from build123d import *

# Parameters (mm, degrees)
YOKE_BODY_DEPTH           = 23
TOP_BLOCK_DEPTH           = 10
TOP_BORE_SKETCH_R         = 8
TOP_BORE_16_DEPTH         = 130.533779378
TOP_COLLAR_SKETCH_R       = 18
TOP_COLLAR_36_DEPTH       = 5
COLLAR_BORE_20_REACH      = 122.147
COLLAR_BORE_SKETCH_R      = 10
SIDE_PIVOT_BOSS_SKETCH_R  = 13
SIDE_PIVOT_BOSS_26_DEPTH  = 19
SIDE_PIVOT_BORE_SKETCH_R  = 6
SIDE_PIVOT_BORE_12_DEPTH  = 130.206230518
SUPPORT_RIB_REACH         = 108.584
SUPPORT_RIB_SKETCH_WALL_W = 247.172853136
SUPPORT_RIB_SKETCH_WALL_H = 10


with BuildPart() as part:
    # Yoke Profile Sketch → Yoke Body (new, symmetric)
    with BuildSketch(Plane.XY):
        with BuildLine():
            Line((19, 10), (-19, 10))
            ThreePointArc((-19, 10), (-21.828427125, 8.828427125), (-23, 6))
            Line((-23, 6), (-23, -21.741149913))
            ThreePointArc((-23, -21.741149913), (-23.246067912, -23.290385113), (-23.960051881, -24.687133484))
            Line((-23.960051881, -24.687133484), (-41.539948119, -48.795166343))
            ThreePointArc((-41.539948119, -48.795166343), (-42.253932088, -50.191914714), (-42.5, -51.741149913))
            Line((-42.5, -51.741149913), (-42.5, -71.741149913))
            Line((-42.5, -71.741149913), (-32.5, -71.741149913))
            Line((-32.5, -71.741149913), (-32.5, -55))
            ThreePointArc((-32.5, -55), (-32.253932088, -53.4507648), (-31.539948119, -52.054016429))
            Line((-31.539948119, -52.054016429), (-15.880155644, -30.579100626))
            ThreePointArc((-15.880155644, -30.579100626), (-13.738203736, -26.388855512), (-13, -21.741149913))
            Line((-13, -21.741149913), (-13, 0))
            Line((-13, 0), (13, 0))
            Line((13, 0), (13, -21.741149913))
            ThreePointArc((13, -21.741149913), (13.738203736, -26.388855512), (15.880155644, -30.579100626))
            Line((15.880155644, -30.579100626), (31.539948119, -52.054016429))
            ThreePointArc((31.539948119, -52.054016429), (32.253932088, -53.4507648), (32.5, -55))
            Line((32.5, -55), (32.5, -71.741149913))
            Line((32.5, -71.741149913), (42.5, -71.741149913))
            Line((42.5, -71.741149913), (42.5, -55))
            ThreePointArc((42.5, -55), (41.761796264, -50.352294401), (39.619844356, -46.162049287))
            Line((39.619844356, -46.162049287), (23.960051881, -24.687133484))
            ThreePointArc((23.960051881, -24.687133484), (23.246067912, -23.290385113), (23, -21.741149913))
            Line((23, -21.741149913), (23, 6))
            ThreePointArc((23, 6), (21.828427125, 8.828427125), (19, 10))
        make_face()
    extrude(amount=YOKE_BODY_DEPTH, both=True)

    # Top Block Sketch → Top Block (add)
    with BuildSketch(Plane(origin=(42.5, 0, 0), x_dir=(0, 0, -1), z_dir=(1, 0, 0))):
        with BuildLine():
            Line((-3, -95), (3, -95))
            ThreePointArc((3, -95), (17.142135624, -89.142135624), (23, -75))
            Line((23, -75), (23, -71.741149913))
            Line((23, -71.741149913), (-23, -71.741149913))
            Line((-23, -71.741149913), (-23, -75))
            ThreePointArc((-23, -75), (-17.142135624, -89.142135624), (-3, -95))
        make_face()
    top_block = extrude(amount=-TOP_BLOCK_DEPTH)

    # Top Block Mirror: Top Block across plane
    add(top_block.mirror(Plane(origin=(0, 0, 0), x_dir=(0, 0, 1), z_dir=(1, 0, 0))))

    # Top Bore Sketch → Top Bore Ø16 (cut, through all)
    with BuildSketch(Plane(origin=(42.5, 0, 0), x_dir=(0, 0, -1), z_dir=(1, 0, 0))):
        with Locations(Location((0, -75, 0), (0, 0, 90))):
            Circle(TOP_BORE_SKETCH_R)
    extrude(amount=-TOP_BORE_16_DEPTH, mode=Mode.SUBTRACT)

    # Top Collar Sketch → Top Collar Ø36 (add)
    with BuildSketch(Plane(origin=(0, 10, 0), x_dir=(1, 0, 0), z_dir=(0, 1, 0))):
        with Locations(Location((0, 0, 0), (0, 0, 90))):
            Circle(TOP_COLLAR_SKETCH_R)
    extrude(amount=TOP_COLLAR_36_DEPTH)

    # Collar Bore Sketch → Collar Bore Ø20 (cut, up to next)
    with BuildSketch(Plane(origin=(0, 15, 0), x_dir=(1, 0, 0), z_dir=(0, 1, 0)), mode=Mode.PRIVATE) as collar_bore_20_sk1:
        with Locations(Location((0, 0, 0), (0, 0, 270))):
            Circle(COLLAR_BORE_SKETCH_R)
    collar_bore_20_tool1 = extrude(collar_bore_20_sk1.sketch, amount=-COLLAR_BORE_20_REACH, mode=Mode.PRIVATE) & part.part
    add(collar_bore_20_tool1.solids().sort_by_distance((0, 15, 0))[0], mode=Mode.SUBTRACT)

    # Side Pivot Boss Sketch → Side Pivot Boss Ø26 (add)
    with BuildSketch(Plane(origin=(23, 0, 0), x_dir=(0, 0, -1), z_dir=(1, 0, 0))):
        with Locations(Location((0, -10, 0), (0, 0, 295.42268723))):
            Circle(SIDE_PIVOT_BOSS_SKETCH_R)
    side_pivot_boss_26 = extrude(amount=SIDE_PIVOT_BOSS_26_DEPTH)

    # Side Pivot Boss Mirror: Side Pivot Boss Ø26 across plane
    add(side_pivot_boss_26.mirror(Plane(origin=(0, 0, 0), x_dir=(0, 0, 1), z_dir=(1, 0, 0))))

    # Side Pivot Bore Sketch → Side Pivot Bore Ø12 (cut, through all)
    with BuildSketch(Plane(origin=(42, 0, 0), x_dir=(0, 0, -1), z_dir=(1, 0, 0))):
        with Locations(Location((0, -10, 0), (0, 0, 270))):
            Circle(SIDE_PIVOT_BORE_SKETCH_R)
    extrude(amount=-SIDE_PIVOT_BORE_12_DEPTH, mode=Mode.SUBTRACT)

    # Support Rib Sketch wall → Support Rib (add, up to next)
    with BuildSketch(Plane(origin=(42.25, -39, 0), x_dir=(0.015623093001, -0.999877952035, 0), z_dir=(0.999877952035, 0.015623093001, 0)), mode=Mode.PRIVATE) as support_rib_sk1:
        Rectangle(SUPPORT_RIB_SKETCH_WALL_W, SUPPORT_RIB_SKETCH_WALL_H)
    support_rib_tool1 = extrude(support_rib_sk1.sketch, amount=-SUPPORT_RIB_REACH, mode=Mode.PRIVATE) - part.part
    support_rib = support_rib_tool1.solids().sort_by_distance((42.25, -39, 0))[0]
    add(support_rib)

    # Support Rib Mirror: Support Rib across plane
    add(support_rib.mirror(Plane(origin=(0, 0, 0), x_dir=(0, 0, 1), z_dir=(1, 0, 0))))


solid = part.part
Here's how the part is built. I have some questions about the finished solid (model axes, mm). A direction names the side the tool comes from. Give positions to 0.01 mm unless a question says otherwise; leave off trailing zeros. Order: outer loops, then holes, each group sorted by start corner. A loop starts at its lowest first (then second) coordinate and runs counter-clockwise, first axis right, second up. Notation, with made-up numbers: (-29.5, 21) -> (-17.5, 21) arc R30 cw to (-17.5, 52) -> close; hole circle Ø9 at (83.25, -26.5). An arc over 180 degrees is marked (long way). One line per item, written item: value. Start each with the question number.
1. Imagine slicing it at A-A, the plane y = -10. List the corners of the cut face in (x, z) for me, plus the area to 3 significant figures.
2. Imagine slicing it at B-B, the plane x = 0. List the corners of the cut face in (y, z) for me.
3. Imagine slicing it at C-C, the plane y = -61. List the corners of the cut face in (x, z) for me.
4. We'd pull the mould along Y, two halves only. Please class faces 5 (the face through (8, 15, -8)), 6 (the face through (32.247, -53.43, 0.322)), 7 (the face through (35, -31, 5)): released by +Y, released by -Y, zero draft, split by the parting line, or undercut.
5. For faces 1 (the face through (-13.76, -26.45, 0.32)), 2 (the face through (23.253, -23.311, 14.126)), 3 (the face through (-35, -30, -5)), 4 (the face through (-23.24, -23.27, 14.13)), which set-ups out of +Z, -Z, +X, -X, +Y, -Y let a thin tool reach every point of the face, with its end or its side?
6. Will these pins go through, and if not, where does the flat tip stop? pin 1 Ø21.5 at (x, y) = (-36, -37.5) entering from -Z; pin 2 Ø12 at (x, z) = (25, -3) entering from +Y; pin 3 Ø14 at (y, z) = (-7, -5) entering from +X; pin 4 Ø24 at (y, z) = (-8.5, -6.5) entering from -X.
7. I need wall thicknesses on probe 1 along Z at (x, y) = (-37, -75); probe 2 along X at (y, z) = (-14, 11); probe 3 along Z at (x, y) = (33, -10). Which ranges of each line are inside material? Lowest first, please. Write a range as from..to.
8. Imagine slicing it at D-D, the plane x = -35. List the corners of the cut face in (y, z) for me, plus the area to 3 significant figures.
Values follow:
1. outline: (-42, -13) -> (-23, -13) -> (-23, -23) -> (-13, -23) -> (-13, -6) -> (-42, -6) -> close; (-42, 6) -> (-13, 6) -> (-13, 23) -> (-23, 23) -> (-23, 13) -> (-42, 13) -> close; (13, -23) -> (23, -23) -> (23, -13) -> (42, -13) -> (42, -6) -> (13, -6) -> close; (13, 6) -> (42, 6) -> (42, 13) -> (23, 13) -> (23, 23) -> (13, 23) -> close
1. area: 1,210 mm2
2. outline: (0, -23) -> (10, -23) -> (10, -18) -> (15, -18) -> (15, -10) -> (0, -10) -> close; (0, 10) -> (15, 10) -> (15, 18) -> (10, 18) -> (10, 23) -> (0, 23) -> close
3. outline: (-42.5, -23) -> (-32.5, -23) -> (-32.5, 23) -> (-42.5, 23) -> close; (32.5, -23) -> (42.5, -23) -> (42.5, 23) -> (32.5, 23) -> close
4. face 5: released by +Y
4. face 6: released by -Y
4. face 7: undercut
5. face 1: +Z, -Z, -Y
5. face 2: +Z, +X
5. face 3: -Z, -X
5. face 4: +Z, -X
6. pin 1: stops at z = -23
6. pin 2: stops at y = 10
6. pin 3: stops at x = 42
6. pin 4: stops at x = -42
7. probe 1: z = -23..-8, 8..23
7. probe 2: x = -42..-13, 13..42
7. probe 3: z = -13..-6, 6..13
8. outline: (-95, -3) arc R20 ccw to (-75, -23) -> (-39.83, -23) -> (-39.83, -5) -> (-22, -5) arc R13 ccw (long way) to (-22, 5) -> (-39.83, 5) -> (-39.83, 23) -> (-75, 23) arc R20 ccw to (-95, 3) -> close; hole circle Ø16 at (-75, 0); hole circle Ø12 at (-10, 0)
8. area: 2,750 mm2
